For this review, take the finished solid that the model builds, in its own axes (mm). A direction names the side the tool comes from. Give positions to 0.01 mm unless a question says otherwise; leave off trailing zeros.
1) For P1, Ø10.5, axis at x = 0, z = 195, coming from the +Y side; P2, Ø9, axis at x = 0, z = -195, coming from the -Y side; P3, Ø8.5, axis at x = 0, z = -175, coming from the +Y side, all flat-tipped, find the tip position at first contact; note any pin that passes through.
2) Draft analysis for pull direction Z (two halves, no side actions). For faces 4 (the face through (0, 3, -215)), 5 (the face through (-5, -7.5, -3)), 6 (the face through (4, 0.7, 175)), state which applies: pulls with the +Z half, pulls with the -Z half, needs draft (parallel to the pull), parting line crosses it, or undercut.
3) Machinability: for faces 1 (the face through (4, 0.7, -175)), 2 (the face through (20, 0, -63)), 3 (the face through (4.4, -4.1, 198.3)), which of the approach directions +Z, -Z, +X, -X, +Y, -Y give a long, thin tool a straight path to every point of the face, cutting with its end or side? Answer none if there is none.
4) Wall thickness on line 1 along Z through (x, y) = (-16.5, -0.5); line 2 along X through (y, z) = (-4, -175); line 3 along Z through (x, y) = (16, -0.25): over which ranges is each line inside the solid? List them lowest first.
from build123d import *

# Parameters (mm, degrees)
SKETCH1_W                                    = 40
SKETCH1_H                                    = 430
BOSS_EXTRUDE1_DEPTH                          = 7.5
SKETCH2_R                                    = 6.5
CUT_EXTRUDE1_DEPTH                           = 3
HEX_SOCKET_CAP_SCREW_HOLE_TYPE_1_D           = 6.6
HEX_SOCKET_CAP_SCREW_HOLE_TYPE_1_CBORE_D     = 11
HEX_SOCKET_CAP_SCREW_HOLE_TYPE_1_CBORE_DEPTH = 6.8
M5_TAPPED_HOLE1_D                            = 4.2
M5_TAPPED_HOLE1_DEPTH                        = 15
M5_TAPPED_HOLE1_TIP                          = 1.2618073
CHAMFER1_SIZE                                = 2
HEX_SOCKET_CAP_SCREW_HOLE_TYPE_2_D           = 6.6
HEX_SOCKET_CAP_SCREW_HOLE_TYPE_2_CBORE_D     = 11
HEX_SOCKET_CAP_SCREW_HOLE_TYPE_2_CBORE_DEPTH = 6.8
M6_TAPPED_HOLE1_D                            = 5
M6_TAPPED_HOLE1_DEPTH                        = 13
M6_TAPPED_HOLE1_TIP                          = 1.502151548
M6_TAPPED_HOLE2_D                            = 5
M6_TAPPED_HOLE2_DEPTH                        = 13
M6_TAPPED_HOLE2_TIP                          = 1.502151548
F_6_0_6_DIAMETER_HOLE1_D                     = 6
F_6_0_6_DIAMETER_HOLE1_DEPTH                 = 17
F_6_0_6_DIAMETER_HOLE1_TIP                   = 1.802581857
SKETCH15_W                                   = 10
SKETCH15_H                                   = 50
CUT_EXTRUDE2_DEPTH                           = 217.448608228
FILLET1_R                                    = 3
CHAMFER2_SIZE                                = 3


with BuildPart() as part:
    # Sketch1 → Boss-Extrude1 (new, symmetric)
    with BuildSketch(Plane(origin=(0, 0, 0), x_dir=(1, 0, 0), z_dir=(0, 1, 0))):
        Rectangle(SKETCH1_W, SKETCH1_H)
    extrude(amount=BOSS_EXTRUDE1_DEPTH, both=True)

    # Sketch2 → Cut-Extrude1 (cut)
    with BuildSketch(Plane(origin=(0, 7.5, 0), x_dir=(1, 0, 0), z_dir=(0, 1, 0))):
        with Locations(Location((0, 195, 0), (0, 0, 270))):
            Circle(SKETCH2_R)
        with Locations(Location((0, -195, 0), (0, 0, 90))):
            Circle(SKETCH2_R)
    extrude(amount=-CUT_EXTRUDE1_DEPTH, mode=Mode.SUBTRACT)

    # Hex socket cap screw hole type 1 (through all)
    with Locations(Plane(origin=(0, -7.5, 0), x_dir=(-1, 0, 0), z_dir=(0, -1, 0))):
        with Locations((0, -195), (0, 195)):
            CounterBoreHole(HEX_SOCKET_CAP_SCREW_HOLE_TYPE_1_D / 2, HEX_SOCKET_CAP_SCREW_HOLE_TYPE_1_CBORE_D / 2, HEX_SOCKET_CAP_SCREW_HOLE_TYPE_1_CBORE_DEPTH)

    # M5 Tapped Hole1
    with Locations(Plane.ZY.offset(20)):
        with Locations((-195, 0), (195, 0), (-65, 0), (65, 0)):
            Hole(M5_TAPPED_HOLE1_D / 2, depth=M5_TAPPED_HOLE1_DEPTH)
            with Locations((0, 0, -(M5_TAPPED_HOLE1_DEPTH + M5_TAPPED_HOLE1_TIP / 2))):  # 118° drill point
                Cone(0, M5_TAPPED_HOLE1_D / 2, M5_TAPPED_HOLE1_TIP, mode=Mode.SUBTRACT)

    # Chamfer1
    chamfer1_edges = [part.edges().sort_by_distance(p)[0] for p in [
        (-20, 0, -215),
        (20, 0, -215),
        (20, 0, 215),
        (-20, 0, 215),
    ]]
    chamfer(chamfer1_edges, length=CHAMFER1_SIZE)

    # Hex socket cap screw hole type 2 (through all)
    with Locations(Plane(origin=(0, 7.5, 0), x_dir=(1, 0, 0), z_dir=(0, 1, 0))):
        with Locations((0, 175), (0, -175), (0, 0)):
            CounterBoreHole(HEX_SOCKET_CAP_SCREW_HOLE_TYPE_2_D / 2, HEX_SOCKET_CAP_SCREW_HOLE_TYPE_2_CBORE_D / 2, HEX_SOCKET_CAP_SCREW_HOLE_TYPE_2_CBORE_DEPTH)

    # M6 Tapped Hole1
    with Locations(Plane.XY.offset(215)):
        with Locations((0, 0)):
            Hole(M6_TAPPED_HOLE1_D / 2, depth=M6_TAPPED_HOLE1_DEPTH)
            with Locations((0, 0, -(M6_TAPPED_HOLE1_DEPTH + M6_TAPPED_HOLE1_TIP / 2))):  # 118° drill point
                Cone(0, M6_TAPPED_HOLE1_D / 2, M6_TAPPED_HOLE1_TIP, mode=Mode.SUBTRACT)

    # M6 Tapped Hole2
    with Locations(Plane(origin=(0, 0, -215), x_dir=(-1, 0, 0), z_dir=(0, 0, -1))):
        with Locations((0, 0)):
            Hole(M6_TAPPED_HOLE2_D / 2, depth=M6_TAPPED_HOLE2_DEPTH)
            with Locations((0, 0, -(M6_TAPPED_HOLE2_DEPTH + M6_TAPPED_HOLE2_TIP / 2))):  # 118° drill point
                Cone(0, M6_TAPPED_HOLE2_D / 2, M6_TAPPED_HOLE2_TIP, mode=Mode.SUBTRACT)

    # Ø6.0 (6) Diameter Hole1
    with Locations(Plane(origin=(0, -7.5, 0), x_dir=(-1, 0, 0), z_dir=(0, -1, 0))):
        with Locations((0, 100), (0, -100)):
            Hole(F_6_0_6_DIAMETER_HOLE1_D / 2, depth=F_6_0_6_DIAMETER_HOLE1_DEPTH)
            with Locations((0, 0, -(F_6_0_6_DIAMETER_HOLE1_DEPTH + F_6_0_6_DIAMETER_HOLE1_TIP / 2))):  # 118° drill point
                Cone(0, F_6_0_6_DIAMETER_HOLE1_D / 2, F_6_0_6_DIAMETER_HOLE1_TIP, mode=Mode.SUBTRACT)

    # Sketch15 → Cut-Extrude2 (cut, through all)
    with BuildSketch(Plane.XZ.offset(7.5)):
        with Locations((15, 110)):
            Rectangle(SKETCH15_W, SKETCH15_H)
    extrude(amount=-CUT_EXTRUDE2_DEPTH, mode=Mode.SUBTRACT)

    # Fillet1
    fillet1_edges = [part.edges().sort_by_distance(p)[0] for p in [
        (10, 0, 85),
        (10, 0, 135),
    ]]
    fillet(fillet1_edges, radius=FILLET1_R)

    # Chamfer2
    chamfer2_edges = [part.edges().sort_by_distance(p)[0] for p in [
        (20, 0, 135),
        (20, 0, 85),
    ]]
    chamfer(chamfer2_edges, length=CHAMFER2_SIZE)


solid = part.part
Results list:
1. P1: stops at y = 4.5
1. P2: stops at y = -0.7
1. P3: stops at y = 0.7
2. face 4: pulls with the -Z half
2. face 5: needs draft
2. face 6: undercut
3. face 1: +Y
3. face 2: +Z, -Z, +X, +Y, -Y
3. face 3: -Y
4. line 1: z = -215 to -197.04, -192.96 to -67.04, -62.96 to 62.96, 67.04 to 192.96, 197.04 to 215
4. line 2: x = -20 to -3.3, 3.3 to 20
4. line 3: z = -215 to 85, 135 to 215
